The model under review builds one solid part; all positions refer to its coordinate system, in mm. A direction names the side the tool comes from. Give positions to 0.01 mm unless a question says otherwise; leave off trailing zeros. Write each loop counter-clockwise with the first axis right and the second up, starting at its lowest first coordinate (ties: lowest second). Pieces come first, ordered by that corner, then holes.
from build123d import *

# Parameters (mm, degrees)
SKETCH_1_R             = 7.5
EXTRUDE_1_DEPTH        = 40
SKETCH_2_W             = 54.950775634
SKETCH_2_H             = 20
CUT_EXTRUDE_1_DEPTH    = 82.547532152
HOLE_WIZARD_M6_1_D     = 5
HOLE_WIZARD_M6_1_DEPTH = 15
HOLE_WIZARD_M6_1_TIP   = 1.502151548


with BuildPart() as part:
    # 草图1 → 凸台-拉伸1 (new body)
    with BuildSketch(Plane(origin=(0, 0, 0), x_dir=(1, 0, 0), z_dir=(0, 1, 0))):
        with BuildLine():
            Line((0, -27.5), (0, 27.5))
            Line((0, 27.5), (10, 27.5))
            Line((10, 27.5), (36.99503609, 13.269117156))
            ThreePointArc((36.99503609, 13.269117156), (45, 0), (36.99503609, -13.269117156))
            Line((36.99503609, -13.269117156), (10, -27.5))
            Line((10, -27.5), (0, -27.5))
        make_face()
        with Locations(Location((30, 0, 0), (0, 0, 270))):
            Circle(SKETCH_1_R, mode=Mode.SUBTRACT)
    extrude(amount=EXTRUDE_1_DEPTH)

    # 草图2 → 切除-拉伸1 (cut, through all)
    with BuildSketch(Plane(origin=(0, 0, -27.5), x_dir=(-1, 0, 0), z_dir=(0, 0, -1))):
        with Locations((-37.475387817, 20)):
            Rectangle(SKETCH_2_W, SKETCH_2_H)
    extrude(amount=-CUT_EXTRUDE_1_DEPTH, mode=Mode.SUBTRACT)

    # M6 螺纹孔1
    with Locations(Plane.ZY):
        with Locations((-19.5, 5), (-19.5, 35), (19.5, 5), (19.5, 35)):
            Hole(HOLE_WIZARD_M6_1_D / 2, depth=HOLE_WIZARD_M6_1_DEPTH)
            with Locations((0, 0, -(HOLE_WIZARD_M6_1_DEPTH + HOLE_WIZARD_M6_1_TIP / 2))):  # 118° drill point
                Cone(0, HOLE_WIZARD_M6_1_D / 2, HOLE_WIZARD_M6_1_TIP, mode=Mode.SUBTRACT)


solid = part.part
1) Tool access review of faces 4 (the flat face through (20, 30, 0)), 5 (the flat face through (18, 0, 0)), 6 (the cylindrical face through (8, 5, 22)): name each direction out of +Z, -Z, +X, -X, +Y, -Y from which nothing blocks a thin tool from reaching the whole face with its end or side.
2) Consider section C-C, the plane x = 30. Give the boundary of the cut face in (y, z).
3) Insertion check: pin 1 (4.5 mm diameter, centred on y = 5, z = 19.5, fed in from +X); pin 2 (1.5 mm diameter, centred on x = 37, y = 34, fed in from +Z); pin 3 (6 mm diameter, centred on y = 16, z = -4, fed in from +X). Each pin has a flat end and moves straight along its axis. Give the tip position at first contact, or say it passes through.
4) Consider section A-A, the plane z = 0. Give the boundary of the cut face in (x, y).
5) The part is to be moulded in two halves that separate along Z. For faces 1 (the flat face through (5, 20, -27.5)), 2 (the conical face through (16.241, 5.293, 19.18)), 3 (the flat face through (5, 20, 27.5)), say which applies: +Z half, -Z half, draft (parallel to the pull), parting line (faces both ways), or undercut.
6) Consider section D-D, the plane z = 23. Give the boundary of the cut face in (x, y), then the cut area to 3 significant figures.
7) Consider section B-B, the plane x = 5. Give the boundary of the cut face in (y, z), then the cut area to 3 significant figures.
8) To check wall thickness, follow probe 1 along Z at (x, y) = (5.5, 5); probe 2 along Y at (x, z) = (23.5, -16.5); probe 3 along X at (y, z) = (3.75, 0). State the ranges of each line that lie inside material, in increasing order.
Answer block:
1. face 4: +Z, -Z, +X
1. face 5: +Z, -Z, +X, -X, -Y
1. face 6: -X
2. outline: (0, -16.96) - (10, -16.96) - (10, -7.5) - (0, -7.5) - close; (0, 7.5) - (10, 7.5) - (10, 16.96) - (0, 16.96) - close; (30, -16.96) - (40, -16.96) - (40, -7.5) - (30, -7.5) - close; (30, 7.5) - (40, 7.5) - (40, 16.96) - (30, 16.96) - close
3. pin 1: stops at x = 29.44
3. pin 2: stops at z = 13.66
3. pin 3: stops at x = 10
4. outline: (0, 0) - (22.5, 0) - (22.5, 10) - (10, 10) - (10, 30) - (22.5, 30) - (22.5, 40) - (0, 40) - close; (37.5, 0) - (45, 0) - (45, 10) - (37.5, 10) - close; (37.5, 30) - (45, 30) - (45, 40) - (37.5, 40) - close
5. face 1: -Z half
5. face 2: undercut
5. face 3: +Z half
6. outline: (0, 0) - (18.54, 0) - (18.54, 10) - (10, 10) - (10, 30) - (18.54, 30) - (18.54, 40) - (0, 40) - close
6. area: 571 mm2
7. outline: (0, -27.5) - (40, -27.5) - (40, 27.5) - (0, 27.5) - close; hole circle Ø5 at (5, -19.5); hole circle Ø5 at (5, 19.5); hole circle Ø5 at (35, -19.5); hole circle Ø5 at (35, 19.5)
7. area: 2,120 mm2
8. probe 1: z = -27.5 to -22, -17 to 17, 22 to 27.5
8. probe 2: y = 0 to 10, 30 to 40
8. probe 3: x = 0 to 22.5, 37.5 to 45
